from build123d import *


with BuildPart() as part:
    # Sketch1 → Revolve1 (revolve)
    with BuildSketch(Plane.XY, mode=Mode.PRIVATE) as revolve1_sk:
        Polygon((0, 0), (0, 100), (4, 100), (4, 115), (11, 115), (21, 97.679491924), (21, 32.5), (39, 27.5), (39, 0), align=None)
    revolve(revolve1_sk.sketch.rotate(Axis((0, 0, 0), (1, 0, 0)), 90), axis=Axis((0, 0, 0), (1, 0, 0)))


solid = part.part
Model file for the job. Use its own axes, mm. A direction names the side the tool comes from. Give positions to 0.01 mm unless a question says otherwise; leave off trailing zeros. Loops run counter-clockwise (first coordinate to the right, second up) from the corner with the lowest first, then second, coordinate; pieces in that order, holes last.
1) Saw through at A-A (y = 0). Write the cut outline in (x, z).
2) Saw through at C-C (x = 7). Write the cut outline in (y, z), plus the area to 3 significant figures.
3) Flat gauge pins, fed straight in: pin 1 Ø6 at (x, y) = (12, -91.5) entering from +Z; pin 2 Ø8 at (x, y) = (8.5, -70) entering from -Z; pin 3 Ø5 at (x, y) = (31, -28.5) entering from +Z; pin 4 Ø12 at (x, y) = (30.5, -71.5) entering from +Z. Where does each tip first touch, or does it go through?
4) Saw through at D-D (x = 35). Write the cut outline in (y, z).
5) Wall check: line 1 (X direction, y = 13, z = 53); line 2 (Y direction, x = 10, z = 18); line 3 (Z direction, x = 15.5, y = -2). Give the ranges that are in metal, low to high.
6) Tool access for faces 1 (the flat face through (21, -23.1, -23.1)), 2 (the flat face through (0, -1, 1)), 3 (the cylindrical face through (2.03, -30.04, 95.38)): list every direction of +Z, -Z, +X, -X, +Y, -Y with a clear straight run to the whole face (end or side of a thin tool).
Answer block:
1. outline: (0, -100) - (4, -100) - (4, -115) - (11, -115) - (21, -97.68) - (21, -32.5) - (39, -27.5) - (39, 27.5) - (21, 32.5) - (21, 97.68) - (11, 115) - (4, 115) - (4, 100) - (0, 100) - close
2. outline: circle Ø230 at (0, 0)
2. area: 41,500 mm2
3. pin 1: stops at z = 73.23
3. pin 2: stops at z = -94.18
3. pin 3: stops at z = 14.62
3. pin 4: passes through
4. outline: circle Ø57.22 at (0, 0)
5. line 1: x = 0 to 21
5. line 2: y = -113.58 to 113.58
5. line 3: z = -107.19 to 107.19
6. face 1: +X
6. face 2: +Z, -Z, -X, +Y, -Y
6. face 3: -X
